The listing builds one solid part. Answer for the finished solid, in the listing's coordinates (mm). Face numbers are marked on the shaded views. A direction names the side the tool comes from. Give positions to 0.01 mm unless a question says otherwise; leave off trailing zeros. Loops run counter-clockwise (first coordinate to the right, second up) from the corner with the lowest first, then second, coordinate; pieces in that order, holes last. Notation, with made-up numbers: M 60.5,-26 L 92.5,-26 A21 cw 92.5,1 Z; hole C 0,81.25 d6. An arc over 180 degrees is marked long. One line per item, written item: value. Start each with the question number.
Q1. Flat-ended cylindrical pins translate along their axes: pin 1 (9 mm diameter, centred on y = -14.5, z = 50, fed in from +X); pin 2 (9.5 mm diameter, centred on x = 36, z = 60, fed in from +Y); pin 3 (4 mm diameter, centred on y = -13.5, z = 43.5, fed in from -X); pin 4 (8 mm diameter, centred on x = 19, y = 6, fed in from +Z). Find the tip coordinate at first contact, or state that the pin passes through.
Q2. A cutting plane is placed at D-D, the plane z = 63.5. Determine the outline of the cut face in (x, y).
Q3. For the marked faces 1, 2, 3 and 4, determine the directions among +Z, -Z, +X, -X, +Y, -Y from which every point of the face is accessible in a straight line to the end or side of a thin tool.
Q4. A cutting plane is placed at B-B, the plane x = 36. Determine the outline of the cut face in (y, z), and give its area (3 significant figures).
Q5. A cutting plane is placed at A-A, the plane y = -19. Determine the outline of the cut face in (x, z).
Q6. Consider L1, parallel to Z at x = 36.5, y = -18.5; L2, parallel to Y at x = 12, z = 4.75; L3, parallel to X at y = -19.5, z = 60. Determine where each line is inside the solid, lowest interval first.
Q7. A cutting plane is placed at C-C, the plane y = 1. Determine the outline of the cut face in (x, z).
Q8. The mould has two halves that part along X. Classify the marked faces 5, 6 and 7: +X half, -X half, draft (parallel to the pull), parting line (faces both ways), or undercut.
from build123d import *

# Parameters (mm, degrees)
MOUNTING_PLATE_DEPTH     = 10
PLATE_NOTCH_SKETCH_W     = 4
PLATE_NOTCH_SKETCH_H     = 5
PLATE_NOTCH_CUT_DEPTH    = 72
PIVOT_ARM_DEPTH          = 8
PIVOT_START              = 5
PIVOT_BOSS_SKETCH_R      = 15
PIVOT_BOSS_30_DEPTH      = 5
PLATE_HOLES_SKETCH_R     = 6
PLATE_HOLES_2X_12_DEPTH  = 10
PIVOT_HOLE_SKETCH_R      = 6
PIVOT_HOLE_12_DEPTH      = 13
GUSSET_BLANK_DEPTH       = 42
GUSSET_TAPER_CUT_DEPTH   = 30
GUSSET_EDGE_TRIM_A_DEPTH = 1
GUSSET_EDGE_TRIM_B_DEPTH = 1


with BuildPart() as part:
    # Plate Profile Sketch → Mounting Plate (new body)
    with BuildSketch(Plane.XY):
        with BuildLine():
            Line((0, 0), (0, -23))
            Line((0, -23), (72, -23))
            Line((72, -23), (72, 0))
            ThreePointArc((72, 0), (68.485281374, 8.485281374), (60, 12))
            Line((60, 12), (12, 12))
            ThreePointArc((12, 12), (3.514718626, 8.485281374), (0, 0))
        make_face()
    extrude(amount=MOUNTING_PLATE_DEPTH)

    # Plate Notch Sketch → Plate Notch Cut (cut)
    with BuildSketch(Plane.ZY):
        with Locations((8, -20.5)):
            Rectangle(PLATE_NOTCH_SKETCH_W, PLATE_NOTCH_SKETCH_H)
    extrude(amount=-PLATE_NOTCH_CUT_DEPTH, mode=Mode.SUBTRACT)

    # Arm Profile Sketch → Pivot Arm (add)
    with BuildSketch(Plane.XZ.offset(18)):
        with BuildLine():
            Line((6, 10), (66, 10))
            ThreePointArc((66, 10), (55.393398282, 14.393398282), (51, 25))
            Line((51, 25), (51, 60))
            ThreePointArc((51, 60), (36, 75), (21, 60))
            Line((21, 60), (21, 25))
            ThreePointArc((21, 25), (16.606601718, 14.393398282), (6, 10))
        make_face()
    extrude(amount=-PIVOT_ARM_DEPTH)

    # Pivot Boss Sketch → Pivot Boss Ø30 (add)
    with BuildSketch(Plane.XZ.offset(18).offset(PIVOT_START)):
        with Locations(Location((36, 60, 0), (0, 0, 270))):
            Circle(PIVOT_BOSS_SKETCH_R)
    extrude(amount=-PIVOT_BOSS_30_DEPTH)

    # Plate Holes Sketch → Plate Holes 2xØ12 (cut)
    with BuildSketch(Plane.XY.offset(10)):
        with Locations((12, 0)):
            Circle(PLATE_HOLES_SKETCH_R)
        with Locations((60, 0)):
            Circle(PLATE_HOLES_SKETCH_R)
    extrude(amount=-PLATE_HOLES_2X_12_DEPTH, mode=Mode.SUBTRACT)

    # Pivot Hole Sketch → Pivot Hole Ø12 (cut)
    with BuildSketch(Plane.XZ.offset(23)):
        with Locations(Location((36, 60, 0), (0, 0, 270))):
            Circle(PIVOT_HOLE_SKETCH_R)
    extrude(amount=-PIVOT_HOLE_12_DEPTH, mode=Mode.SUBTRACT)

    # Gusset Profile Sketch → Gusset Blank (add)
    with BuildSketch(Plane.ZY):
        Polygon((10, -10), (50.245930421, -10), (10, 12), align=None)
    extrude(amount=-GUSSET_BLANK_DEPTH)

    # Gusset Taper Sketch → Gusset Taper Cut (cut)
    with BuildSketch(Plane.ZY):
        Polygon((10, 12), (10, -10), (50.245930421, -10), align=None)
    extrude(amount=-GUSSET_TAPER_CUT_DEPTH, mode=Mode.SUBTRACT)

    # Gusset Edge Trim A Sketch → Gusset Edge Trim A (cut)
    with BuildSketch(Plane.ZY.offset(-30)):
        Polygon((10, 12), (10, -10), (50.245930421, -10), align=None)
    extrude(amount=-GUSSET_EDGE_TRIM_A_DEPTH, mode=Mode.SUBTRACT)

    # Gusset Edge Trim B Sketch → Gusset Edge Trim B (cut)
    with BuildSketch(Plane(origin=(42, 0, 0), x_dir=(0, 0, -1), z_dir=(1, 0, 0))):
        Polygon((-50.245930421, -10), (-10, -10), (-10, 12), align=None)
    extrude(amount=-GUSSET_EDGE_TRIM_B_DEPTH, mode=Mode.SUBTRACT)


solid = part.part
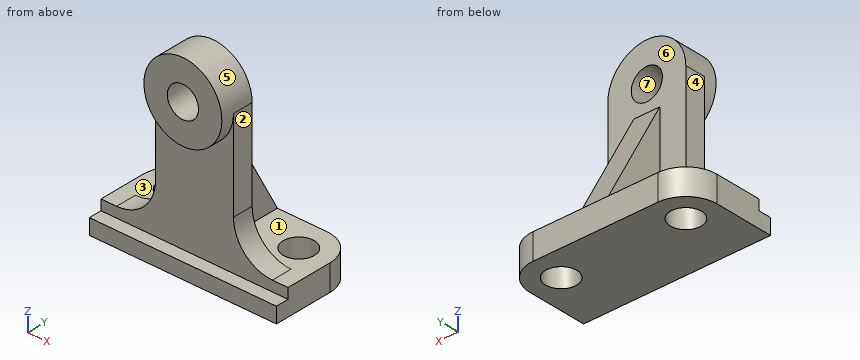
Answer block:
1. pin 1: x = 51
1. pin 2: through
1. pin 3: x = 21
1. pin 4: z = 10
2. outline: M 21.41,-23 L 31.13,-23 L 31.13,-10 L 21.41,-10 Z; M 40.87,-23 L 50.59,-23 L 50.59,-10 L 40.87,-10 Z
3. face 1: +Z, +X, +Y
3. face 2: +Z, +X, +Y, -Y
3. face 3: +Z, -X, +Y
3. face 4: +Z, -X, +Y, -Y
4. outline: M -23,0 L 12,0 L 12,10 L -10,50.25 L -10,54 L -23,54 L -23,45 L -18,45 L -18,6 L -23,6 Z; M -23,66 L -10,66 L -10,75 L -23,75 Z
4. area: 1,290 mm^2
5. outline: M 0,0 L 72,0 L 72,6 L 0,6 Z; C 36,60 d30; hole C 36,60 d12
6. L1: 0 to 6, 45.01 to 54.02, 65.98 to 74.99
6. L2: -23 to -6, 6 to 12
6. L3: 21 to 30, 42 to 51
7. outline: M 0.04,0 L 6.08,0 L 6.08,10 L 0.04,10 Z; M 17.92,0 L 54.08,0 L 54.08,10 L 41,10 L 41,30.12 L 31,30.12 L 31,10 L 17.92,10 Z; M 65.92,0 L 71.96,0 L 71.96,10 L 65.92,10 Z
8. face 5: parting line
8. face 6: draft
8. face 7: undercut
